CAD build for the part. Positions are in the model's coordinates, mm. Coordinates: 2 decimals unless noted, no trailing zeros. Loops run counter-clockwise (first coordinate to the right, second up) from the corner with the lowest first, then second, coordinate; pieces in that order, holes last. Notation, with made-up numbers: M -39,83 L -12,83 A36 cw -12,118 Z; hole C 84.5,32 d8. An arc over 180 degrees is marked long. Answer as a JSON object with one key per item and string values. Group by question number.
```python
from build123d import *

# Parameters (mm, degrees)
SKETCH1_W           = 115
SKETCH1_H           = 30
SKETCH1_R           = 3.25
BOSS_EXTRUDE1_DEPTH = 4
CHAMFER1_SIZE       = 2


with BuildPart() as part:
    # Sketch1 → Boss-Extrude1 (new body)
    with BuildSketch(Plane.XY):
        Rectangle(SKETCH1_W, SKETCH1_H)
        with Locations((-37.5, 0)):
            Circle(SKETCH1_R, mode=Mode.SUBTRACT)
        with Locations((37.5, 0)):
            Circle(SKETCH1_R, mode=Mode.SUBTRACT)
    extrude(amount=BOSS_EXTRUDE1_DEPTH)

    # Chamfer1
    chamfer1_edges = [part.edges().sort_by_distance(p)[0] for p in [
        (-57.5, 15, 2),
        (57.5, 15, 2),
        (57.5, -15, 2),
        (-57.5, -15, 2),
    ]]
    chamfer(chamfer1_edges, length=CHAMFER1_SIZE)


solid = part.part
```
Item 1: Slice it at C-C, the plane z = 1.4. Write the cut outline in (x, y), then the cut area to 3 significant figures.
Item 2: Pull direction X, two halves, no side cores. Call faces 1 (the cylindrical face through (-34.498, -1.245, 1.972)), 2 (the flat face through (-56.5, 14, 2)), 3 (the flat face through (-1, 0, 4)): released by +X, released by -X, zero draft, split by the parting line, or undercut.
Item 3: Slice it at A-A, the plane y = 0. Write the cut outline in (x, z).
Item 4: Drill centre lines: L1, parallel to X at y = -0.25, z = 1.8; L2, parallel to Y at x = 37.5, z = 2.5; L3, parallel to X at y = -2.5, z = 1.25. Where is each one in solid material? Low to high. Write a range as from..to.
Item 5: Slice it at B-B, the plane x = -37.5. Write the cut outline in (y, z).
Computed:
{
 "1": {"outline": "M -57.5,-13 L -55.5,-15 L 55.5,-15 L 57.5,-13 L 57.5,13 L 55.5,15 L -55.5,15 L -57.5,13 Z; hole C -37.5,0 d6.5; hole C 37.5,0 d6.5", "area": "3,380 mm2"},
 "2": {"face 1": "undercut", "face 2": "released by -X", "face 3": "zero draft"},
 "3": {"outline": "M -57.5,0 L -40.75,0 L -40.75,4 L -57.5,4 Z; M -34.25,0 L 34.25,0 L 34.25,4 L -34.25,4 Z; M 40.75,0 L 57.5,0 L 57.5,4 L 40.75,4 Z"},
 "4": {"L1": "-57.5..-40.74, -34.26..34.26, 40.74..57.5", "L2": "-15..-3.25, 3.25..15", "L3": "-57.5..-39.58, -35.42..35.42, 39.58..57.5"},
 "5": {"outline": "M -15,0 L -3.25,0 L -3.25,4 L -15,4 Z; M 3.25,0 L 15,0 L 15,4 L 3.25,4 Z"}
}
